Here's how the part is built. I have some questions about the finished solid (model axes, mm). Face numbers are marked on the shaded views. A direction names the side the tool comes from. Give positions to 0.01 mm unless a question says otherwise; leave off trailing zeros. Loops run counter-clockwise (first coordinate to the right, second up) from the corner with the lowest first, then second, coordinate; pieces in that order, holes last. Notation, with made-up numbers: M -5.5,-36 L 21.5,-36 A16 cw 21.5,-11 Z; hole C 25,-29.5 d10. An arc over 180 degrees is marked long. Answer as CSV lines item,"result". Start each with the question number.
Item 1: I want a section at A-A on z = 7.25. List the corners of the cut face in (x, y) for me, plus the area to 3 significant figures.
Item 2: For the marked faces 1, 2 and 3, which set-ups out of +Z, -Z, +X, -X, +Y, -Y let a thin tool reach every point of the face, with its end or its side?
Item 3: I want a section at B-B on z = 15.75. List the corners of the cut face in (x, y) for me, plus the area to 3 significant figures.
Item 4: If I drill on line 1 along X through (y, z) = (-2, 5.75); line 2 along Y through (x, z) = (0, 14.25); line 3 along X through (y, z) = (1, 15.25), over which ranges is the centre line in solid material (lowest first)? Write a range as from..to.
Item 5: Will these pins go through, and if not, where does the flat tip stop? P1, Ø1, axis at x = 2.5, y = -2, coming from the -Z side; P2, Ø0.6, axis at x = -2, y = -0.5, coming from the +Z side; P3, Ø1, axis at x = -2.5, y = -2.5, coming from the -Z side.
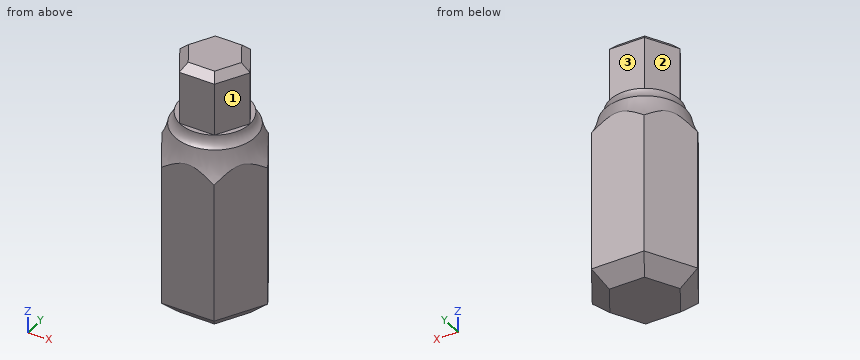
from build123d import *

# Parameters (mm, degrees)
HEX_SHANK_6AF_X13_DEPTH   = 13
HEX_TIP_4AF_X4_DEPTH      = 4
HEX_TIP_4AF_X4_DEPTH_BACK = 4
TIP_CHAMFER_0_5_SIZE      = 0.5
SHANK_CHAMFER_1_SIZE      = 1


with BuildPart() as part:
    # Hex Shank Profile 6AF → Hex Shank 6AF x13 (new body)
    with BuildSketch(Plane.XY):
        Polygon((3.464101615, 0), (1.732050808, 3), (-1.732050808, 3), (-3.464101615, 0), (-1.732050808, -3), (1.732050808, -3), align=None)
    extrude(amount=HEX_SHANK_6AF_X13_DEPTH)

    # Hex Tip Profile 4AF → Hex Tip 4AF x4 (add, two sides: drawn at the far end of the back side and taken through both)
    with BuildSketch(Plane.XY.offset(13).offset(-HEX_TIP_4AF_X4_DEPTH_BACK)):
        Polygon((2.309401077, 0), (1.154700538, 2), (-1.154700538, 2), (-2.309401077, 0), (-1.154700538, -2), (1.154700538, -2), align=None)
    extrude(amount=HEX_TIP_4AF_X4_DEPTH + HEX_TIP_4AF_X4_DEPTH_BACK)

    # Neck Groove Profile → Neck Groove (revolve, cut)
    with BuildSketch(Plane(origin=(0, 0, 0), x_dir=(1, 0, 0), z_dir=(0, 1, 0)), mode=Mode.PRIVATE) as neck_groove_sk:
        with BuildLine():
            Line((3.464101615, -10.360098242), (3.464101615, -13))
            Line((3.464101615, -13), (2.309401077, -13))
            ThreePointArc((2.309401077, -13), (2.40550356, -12.572250915), (2.675339636, -12.226717329))
            ThreePointArc((2.675339636, -12.226717329), (2.963282684, -11.248431174), (3.464101615, -10.360098242))
        make_face()
    revolve(neck_groove_sk.sketch.rotate(Axis((0, 0, 0), (0, 0, 1)), 180), axis=Axis((0, 0, 0), (0, 0, 1)), mode=Mode.SUBTRACT)

    # Tip Chamfer 0.5
    tip_chamfer_0_5_edges = [part.edges().sort_by_distance(p)[0] for p in [
        (1.732050808, -1, 17),
        (1.732050808, 1, 17),
        (0, 2, 17),
        (-1.732050808, 1, 17),
        (-1.732050808, -1, 17),
        (0, -2, 17),
    ]]
    chamfer(tip_chamfer_0_5_edges, length=TIP_CHAMFER_0_5_SIZE)

    # Shank Chamfer 1
    shank_chamfer_1_edges = [part.edges().sort_by_distance(p)[0] for p in [
        (0, -3, 0),
        (-2.598076211, -1.5, 0),
        (-2.598076211, 1.5, 0),
        (0, 3, 0),
        (2.598076211, 1.5, 0),
        (2.598076211, -1.5, 0),
    ]]
    chamfer(shank_chamfer_1_edges, length=SHANK_CHAMFER_1_SIZE)


solid = part.part
Result:
1,outline,"M -3.46,0 L -1.73,-3 L 1.73,-3 L 3.46,0 L 1.73,3 L -1.73,3 Z"
1,area,"31.2 mm^2"
2,face 1,"+Z, +X, -Y"
2,face 2,"+Z, -X, +Y"
2,face 3,"+Z, +X, -X, +Y"
3,outline,"M -2.31,0 L -1.15,-2 L 1.15,-2 L 2.31,0 L 1.15,2 L -1.15,2 Z"
3,area,"13.9 mm^2"
4,line 1,"-2.31..2.31"
4,line 2,"-2..2"
4,line 3,"-1.73..1.73"
5,P1,"z = 0.67"
5,P2,"z = 16.82"
5,P3,"z = 0.92"
